from build123d import *

# Parameters (mm, degrees)
SKETCH_1_W             = 58
SKETCH_1_H             = 90
EXTRUDE_1_DEPTH        = 7.5
HOLE_WIZARD_M8_1_D     = 6.8
HOLE_WIZARD_M8_1_DEPTH = 19.75
HOLE_WIZARD_M8_1_TIP   = 2.042926105
M20X1_5_1_D            = 18.5
M20X1_5_1_DEPTH        = 44.5
M20X1_5_1_TIP          = 5.557960726
CHAMFER_1_SIZE         = 5


with BuildPart() as part:
    # 草图1 → 凸台-拉伸1 (new, symmetric)
    with BuildSketch(Plane(origin=(0, 0, 0), x_dir=(1, 0, 0), z_dir=(0, 1, 0))):
        Rectangle(SKETCH_1_W, SKETCH_1_H)
    extrude(amount=EXTRUDE_1_DEPTH, both=True)

    # M8 螺纹孔1
    with Locations(Plane.XZ.offset(7.5)):
        with Locations((-22.5, -32.5), (22.5, -32.5), (22.5, 32.5), (-22.5, 32.5)):
            Hole(HOLE_WIZARD_M8_1_D / 2, depth=HOLE_WIZARD_M8_1_DEPTH)
            with Locations((0, 0, -(HOLE_WIZARD_M8_1_DEPTH + HOLE_WIZARD_M8_1_TIP / 2))):  # 118° drill point
                Cone(0, HOLE_WIZARD_M8_1_D / 2, HOLE_WIZARD_M8_1_TIP, mode=Mode.SUBTRACT)

    # M20x1.5 螺纹孔1
    with Locations(Plane(origin=(0, 7.5, 0), x_dir=(1, 0, 0), z_dir=(0, 1, 0))):
        with Locations((0, 0)):
            Hole(M20X1_5_1_D / 2, depth=M20X1_5_1_DEPTH)
            with Locations((0, 0, -(M20X1_5_1_DEPTH + M20X1_5_1_TIP / 2))):  # 118° drill point
                Cone(0, M20X1_5_1_D / 2, M20X1_5_1_TIP, mode=Mode.SUBTRACT)

    # 倒角1
    chamfer_1_edges = [part.edges().sort_by_distance(p)[0] for p in [
        (29, 0, 45),
        (-29, 0, 45),
        (-29, 0, -45),
        (29, 0, -45),
    ]]
    chamfer(chamfer_1_edges, length=CHAMFER_1_SIZE)


solid = part.part
Geometry: final body of the model. Coordinates: model frame, mm. Give positions to 0.01 mm unless a question says otherwise; leave off trailing zeros. Loops run counter-clockwise (first coordinate to the right, second up) from the corner with the lowest first, then second, coordinate; pieces in that order, holes last. Notation, with made-up numbers: (86, -14.5) - (110, -14.5) arc R16 cw to (110, 5.5) - close; hole circle Ø10 at (21.25, 22.25). An arc over 180 degrees is marked (long way). One line per question, with ' | ' between items. Start each with the question number.
(1) Section query B-B on z = 0. Return loops of the section in (x, y), then the cut area to 4 significant figures.
(2) Pull-direction query (Z, two-part tool) for faces 1 (the cylindrical face through (2.01, -0.11, 9.03)), 2 (the flat face through (-0.4, -7.5, 9.4)), 3 (the flat face through (27, 0, 42)); classes: released by +Z, released by -Z, zero draft, split by the parting line, or undercut.
(3) Section query A-A on z = -32.5. Return loops of the section in (x, y).
(4) Ray query, line 1 (Z direction, x = 22.5, y = -1); line 2 (Z direction, x = 23.5, y = 3.25); line 3 (X direction, y = -6, z = -6). Return the intervals inside material, ascending. Write a range as from..to.
(5) Contact query for flat-ended pins moving along their axis: pin 1 (11 mm diameter, centred on x = 22.5, z = -32.5, fed in from +Y); pin 2 (6 mm diameter, centred on x = 22.5, z = 32.5, fed in from -Y). Output: stop coordinate, or through.
(6) Section query D-D on x = -22.5. Return loops of the section in (y, z), then the cut area to 3 significant figures.
(7) Section query C-C on x = 0. Return loops of the section in (y, z).
The answers:
1) outline: (-29, -7.5) - (-9.25, -7.5) - (-9.25, 7.5) - (-29, 7.5) - close; (9.25, -7.5) - (29, -7.5) - (29, 7.5) - (9.25, 7.5) - close | area: 592.5 mm2
2) face 1: undercut | face 2: zero draft | face 3: released by +Z
3) outline: (-29, -7.5) - (-25.9, -7.5) - (-25.9, 7.5) - (-29, 7.5) - close; (-19.1, -7.5) - (19.1, -7.5) - (19.1, 7.5) - (-19.1, 7.5) - close; (25.9, -7.5) - (29, -7.5) - (29, 7.5) - (25.9, 7.5) - close
4) line 1: -45..-35.9, -29.1..29.1, 35.9..45 | line 2: -45..-35.75, -29.25..29.25, 35.75..45 | line 3: -29..-7.04, 7.04..29
5) pin 1: y = 7.5 | pin 2: through
6) outline: (-7.5, -45) - (7.5, -45) - (7.5, -35.9) - (-7.5, -35.9) - close; (-7.5, -29.1) - (7.5, -29.1) - (7.5, 29.1) - (-7.5, 29.1) - close; (-7.5, 35.9) - (7.5, 35.9) - (7.5, 45) - (-7.5, 45) - close | area: 1,150 mm2
7) outline: (-7.5, -45) - (7.5, -45) - (7.5, -9.25) - (-7.5, -9.25) - close; (-7.5, 9.25) - (7.5, 9.25) - (7.5, 45) - (-7.5, 45) - close
